from build123d import *

# Parameters (mm, degrees)
SKETCH1_W           = 150
SKETCH1_H           = 40
SKETCH1_R           = 12
BOSS_EXTRUDE1_DEPTH = 10
FILLET1_R           = 10


with BuildPart() as part:
    # Sketch1 → Boss-Extrude1 (new body)
    with BuildSketch(Plane.XY):
        Rectangle(SKETCH1_W, SKETCH1_H)
        with Locations((50, 0)):
            Circle(SKETCH1_R, mode=Mode.SUBTRACT)
        with Locations((-50, 0)):
            Circle(SKETCH1_R, mode=Mode.SUBTRACT)
    extrude(amount=BOSS_EXTRUDE1_DEPTH)

    # Fillet1
    fillet1_edges = [part.edges().sort_by_distance(p)[0] for p in [
        (75, -20, 5),
        (-75, -20, 5),
        (-75, 20, 5),
        (75, 20, 5),
    ]]
    fillet(fillet1_edges, radius=FILLET1_R)


solid = part.part
Work out the finished part from the listing and answer in its coordinate system (mm). Give positions to 0.01 mm unless a question says otherwise; leave off trailing zeros. Order: outer loops, then holes, each group sorted by start corner. A loop starts at its lowest first (then second) coordinate and runs counter-clockwise, first axis right, second up. Notation, with made-up numbers: M -35.75,-11 L 9.25,-11 A19 cw 9.25,1 Z; hole C 72.5,-33 d4. An arc over 180 degrees is marked long. Return JSON: item names as keys, results as strings.
Q1. This flat-tipped pin is pushed along its axis until it touches: pin 1 (14.5 mm diameter, centred on x = -50, y = 0, fed in from -Z). Where does it stop, or does it pass through?
Answer below:
{"pin 1": "passes through"}
Q2. Find section A-A, the plane y = 0. Write down the section's boundary in (x, z), and give its area (3 significant figures).
Answer below:
{"outline": "M -75,0 L -62,0 L -62,10 L -75,10 Z; M -38,0 L 38,0 L 38,10 L -38,10 Z; M 62,0 L 75,0 L 75,10 L 62,10 Z", "area": "1,020 mm^2"}
Q3. Find the intervals of material crossed by line 1 along X through (y, z) = (-6, 8); line 2 along X through (y, z) = (2, 9.5); line 3 along Y through (x, z) = (-50, 4.5), in increasing order. Write a range as [from, to].
Answer below:
{"line 1": "x = [-75, -60.39], [-39.61, 39.61], [60.39, 75]", "line 2": "x = [-75, -61.83], [-38.17, 38.17], [61.83, 75]", "line 3": "y = [-20, -12], [12, 20]"}
Q4. Find section B-B, the plane x = -50. Write down the section's boundary in (y, z).
Answer below:
{"outline": "M -20,0 L -12,0 L -12,10 L -20,10 Z; M 12,0 L 20,0 L 20,10 L 12,10 Z"}
Q5. Find section C-C, the plane z = 4. Write down the section's boundary in (x, y).
Answer below:
{"outline": "M -75,-10 A10 ccw -65,-20 L 65,-20 A10 ccw 75,-10 L 75,10 A10 ccw 65,20 L -65,20 A10 ccw -75,10 Z; hole C -50,0 d24; hole C 50,0 d24"}
Q6. Find section D-D, the plane y = 8.5. Write down the section's boundary in (x, z), and give its area (3 significant figures).
Answer below:
{"outline": "M -75,0 L -58.47,0 L -58.47,10 L -75,10 Z; M -41.53,0 L 41.53,0 L 41.53,10 L -41.53,10 Z; M 58.47,0 L 75,0 L 75,10 L 58.47,10 Z", "area": "1,160 mm^2"}
Q7. The mould has two halves that part along X. Classify faces 1 (the face through (-59.523, -7.302, 4.93)), 2 (the face through (71.99, -17.15, 5.07)), 3 (the face through (-72.15, -16.99, 5.07)): pulls with the +X half, pulls with the -X half, needs draft (parallel to the pull), parting line crosses it, or undercut.
Answer below:
{"face 1": "undercut", "face 2": "pulls with the +X half", "face 3": "pulls with the -X half"}
